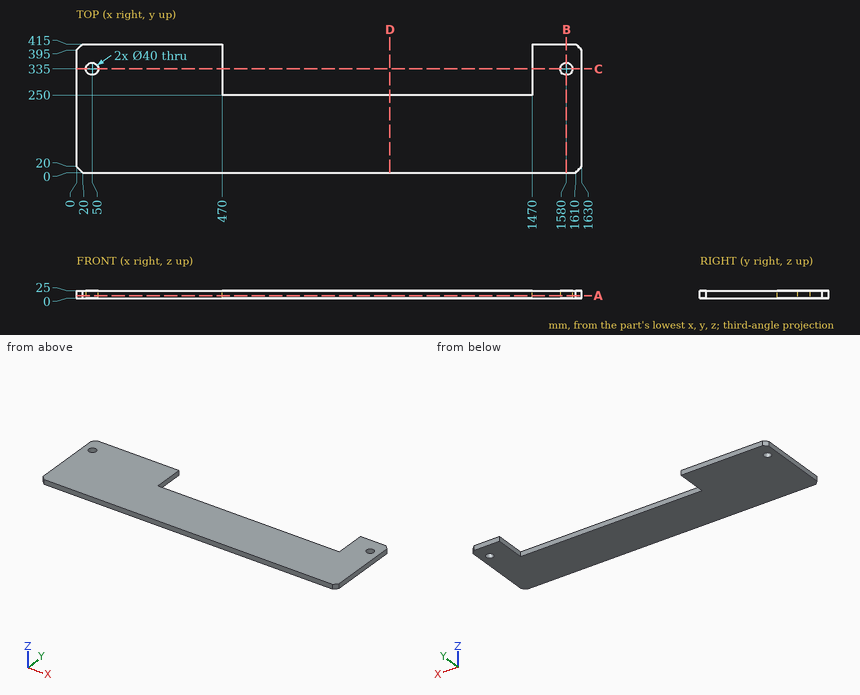
Geometry check sheet. Reference: drawing and pictorial views, mm from the part's lowest x, y, z. Coordinates: 2 decimals unless noted, no trailing zeros. Order: outer loops, then holes, each group sorted by start corner. A loop starts at its lowest first (then second) coordinate and runs counter-clockwise, first axis right, second up. Notation, with made-up numbers: (71.25, -21) - (97.25, -21) arc R23 cw to (97.25, 3) - close; hole circle Ø7 at (10, -1.75). An arc over 180 degrees is marked (long way). Answer in a Markdown table with one row per item. Add a question column.
1) Cross-section at C-C, the plane y = 335. Record the cut outline in (x, z).
2) Cross-section at A-A, the plane z = 8.75. Record the cut outline in (x, y), then the cut area to 3 significant figures.
3) Cross-section at B-B, the plane x = 1580. Record the cut outline in (y, z).
4) Material ranges on line 1 along X through (y, z) = (335, 11.25); line 2 along Y through (x, z) = (1580, 15.5); line 3 along X through (y, z) = (369, 15.5), recorded low to high. Write a range as [from, to].
5) Gauge pin test, flat end, axial feed: P1, Ø3, axis at x = 857, z = 6, coming from the +Y side. Record the tip position at first contact, or that the pin passes through.
6) Cross-section at D-D, the plane x = 1011. Record the cut outline in (y, z).
Check result:
| question | item | result |
|---|---|---|
| 1 | outline | (0, 0) - (30, 0) - (30, 25) - (0, 25) - close; (70, 0) - (470, 0) - (470, 25) - (70, 25) - close; (1470, 0) - (1560, 0) - (1560, 25) - (1470, 25) - close; (1600, 0) - (1630, 0) - (1630, 25) - (1600, 25) - close |
| 2 | outline | (0, 20) - (20, 0) - (1610, 0) - (1630, 20) - (1630, 395) - (1610, 415) - (1470, 415) - (1470, 250) - (470, 250) - (470, 415) - (20, 415) - (0, 395) - close; hole circle Ø40 at (50, 335); hole circle Ø40 at (1580, 335) |
| 2 | area | 508,000 mm² |
| 3 | outline | (0, 0) - (315, 0) - (315, 25) - (0, 25) - close; (355, 0) - (415, 0) - (415, 25) - (355, 25) - close |
| 4 | line 1 | x = [0, 30], [70, 470], [1470, 1560], [1600, 1630] |
| 4 | line 2 | y = [0, 315], [355, 415] |
| 4 | line 3 | x = [0, 470], [1470, 1630] |
| 5 | P1 | stops at y = 250 |
| 6 | outline | (0, 0) - (250, 0) - (250, 25) - (0, 25) - close |
